Build history of the part. All positions in model axes, mm. A direction names the side the tool comes from. Round coordinates to 2 decimals unless told otherwise and drop trailing zeros. Loops run counter-clockwise (first coordinate to the right, second up) from the corner with the lowest first, then second, coordinate; pieces in that order, holes last. Notation, with made-up numbers: (-19, 67) -> (1, 67) arc R32 cw to (1, 104) -> close; hole circle Ø8 at (75, 46.25). An arc over 180 degrees is marked (long way). Put each result on its own line as item: value. Start each with the question number.
Item 1: Pull direction X, two halves, no side cores. Call faces 1 (the flat face through (-60.136, 53, -48)), 2 (the flat face through (-30.136, 48, -42)), 3 (the cylindrical face through (-15.556, 87.485, -73.11)), 4 (the cylindrical face through (-40, 45.05, -38.12)): +X half, -X half, draft (parallel to the pull), parting line (faces both ways), or undercut.
Item 2: Cut at B-B, the plane y = 87. List the corners of the cut face in (x, z), plus the area to 3 significant figures.
Item 3: Cut at D-D, the plane y = 70. List the corners of the cut face in (x, z), plus the area to 3 significant figures.
Item 4: Drill centre lines: probe 1 along X at (y, z) = (105.5, -31.5); probe 2 along X at (y, z) = (22, -84.5); probe 3 along X at (y, z) = (69, -49). Where is each one in solid material? Low to high. Write a range as [from, to].
Item 5: Tool access for faces 5 (the flat face through (-31.18, 14.42, -89.05)), 6 (the cylindrical face through (-14.926, 82.124, -68.609)), 7 (the cylindrical face through (9.93, 48.87, -41.35)), 8 (the cylindrical face through (-55.066, 61.239, -53.737)), 9 (the cylindrical face through (-15.626, 91.391, -76.232)): list every direction of +Z, -Z, +X, -X, +Y, -Y with a clear straight run to the whole face (end or side of a thin tool).
Item 6: Cut at A-A, the plane x = -40.5. List the corners of the cut face in (y, z), plus the area to 3 significant figures.
Item 7: Flat gauge pins, fed straight in: pin 1 Ø1.5 at (x, z) = (6, -24) entering from -Y; pin 2 Ø4 at (x, z) = (-26.5, -29) entering from +Y; pin 3 Ø10 at (x, z) = (7, -74.5) entering from -Y. Where does each tip first touch, or does it go through?
Item 8: Cut at C-C, the plane z = -96.5. List the corners of the cut face in (x, y), plus the area to 3 significant figures.
```python
from build123d import *

# Parameters (mm, degrees)
REVOLVE1_ANGLE                 = 80
SKETCH3_R                      = 7.5
BOSS_EXTRUDE1_DEPTH            = 10
SHELL3_T                       = -5
CUT_EXTRUDE1_REACH             = 176.812
SKETCH4_R                      = 15
CUT_EXTRUDE1_DIRECTION_2_REACH = 176.812


with BuildPart() as part:
    # Sketch1 → Revolve1 (revolve)
    with BuildSketch(Plane.XY):
        Polygon((-0.136394071, 58.716551136), (19.863605929, 58.716551136), (19.863605929, 118.716551136), (-50.136394071, 118.716551136), (-50.136394071, 58.716551136), (-30.136394071, 58.716551136), (-30.136394071, 106.716551136), (-0.136394071, 106.716551136), align=None)
    revolve(axis=Axis((39.541450035, -1.283448864, 0), (-1, 0, 0)), revolution_arc=REVOLVE1_ANGLE)

    # Sketch3 → Boss-Extrude1 (add)
    with BuildSketch(Plane.ZY.offset(50.136394071)):
        with Locations((-48.209070726, 56.16988437)):
            Circle(SKETCH3_R)
    extrude(amount=BOSS_EXTRUDE1_DEPTH)

    # Shell3
    shell3_openings = [part.faces().sort_by_distance(p)[0] for p in [
        (-60.136394071, 56.16988437, -48.209070726),
    ]]
    offset(amount=SHELL3_T, openings=shell3_openings, kind=Kind.INTERSECTION)

    # Sketch4 → Cut-Extrude1 (cut, up to next)
    with BuildSketch(Plane(origin=(-30.136394071, 0, 0), x_dir=(0, 0, -1), z_dir=(1, 0, 0)), mode=Mode.PRIVATE) as cut_extrude1_sk1:
        with Locations(Location((52.708583994, 61.532195472, 0), (0, 0, 270))):
            Circle(SKETCH4_R)
    cut_extrude1_tool1 = extrude(cut_extrude1_sk1.sketch, amount=-CUT_EXTRUDE1_REACH, mode=Mode.PRIVATE) & part.part
    add(cut_extrude1_tool1.solids().sort_by_distance((-30.136394, 61.532195, -52.708584))[0], mode=Mode.SUBTRACT)

    # Sketch4 → Cut-Extrude1 direction 2 (cut, up to next)
    with BuildSketch(Plane(origin=(-30.136394071, 0, 0), x_dir=(0, 0, -1), z_dir=(1, 0, 0)), mode=Mode.PRIVATE) as cut_extrude1_direction_2_sk1:
        with Locations(Location((52.708583994, 61.532195472, 0), (0, 0, 270))):
            Circle(SKETCH4_R)
    cut_extrude1_direction_2_tool1 = extrude(cut_extrude1_direction_2_sk1.sketch, amount=CUT_EXTRUDE1_DIRECTION_2_REACH, mode=Mode.PRIVATE) & part.part
    add(cut_extrude1_direction_2_tool1.solids().sort_by_distance((-30.136394, 61.532195, -52.708584))[0], mode=Mode.SUBTRACT)


solid = part.part
```
Reply:
1. face 1: -X half
1. face 2: undercut
1. face 3: undercut
1. face 4: draft
2. outline: (-50.14, -81.28) -> (19.86, -81.28) -> (19.86, 0) -> (-0.14, 0) -> (-0.14, -62.21) -> (-30.14, -62.21) -> (-30.14, 0) -> (-50.14, 0) -> close; hole (-45.14, -73.7) -> (14.86, -73.7) -> (14.86, -5) -> (4.86, -5) -> (4.86, -70.53) -> (-35.14, -70.53) -> (-35.14, -5) -> (-45.14, -5) -> close
2. area: 2,320 mm^2
3. outline: (-50.14, -96.53) -> (19.86, -96.53) -> (19.86, 0) -> (-0.14, 0) -> (-0.14, -40.33) -> (4.86, -40.33) -> (4.86, -5) -> (14.86, -5) -> (14.86, -90.24) -> (-45.14, -90.24) -> (-45.14, -5) -> (-35.14, -5) -> (-35.14, -40.33) -> (-30.14, -40.33) -> (-30.14, 0) -> (-50.14, 0) -> close; (-35.14, -87.68) -> (4.86, -87.68) -> (4.86, -65.09) -> (-0.14, -65.09) -> (-0.14, -81.13) -> (-30.14, -81.13) -> (-30.14, -65.09) -> (-35.14, -65.09) -> close
3. area: 2,270 mm^2
4. probe 1: x = [-50.14, -45.14], [-35.14, 4.86], [14.86, 19.86]
4. probe 2: x = [-50.14, -45.14], [-35.14, -30.14], [-0.14, 4.86], [14.86, 19.86]
4. probe 3: x = [-50.14, -45.14], [14.86, 19.86]
5. face 5: -Z, +X, -X, -Y
5. face 6: +Z, -Y
5. face 7: none
5. face 8: -X
5. face 9: -Z, +X, -X, +Y
6. outline: (9.14, -59.09) -> (19.55, -118.18) arc R120 ccw to (118.72, 0) -> (58.72, 0) arc R60 cw to start; hole (14.89, -62.95) -> (23.59, -112.28) arc R115 ccw to (113.61, -5) -> (63.52, -5) arc R65 cw to start
6. area: 1,760 mm^2
7. pin 1: stops at y = 53.37
7. pin 2: stops at y = 115.64
7. pin 3: stops at y = 10.97
8. outline: (-50.14, 15.73) -> (-30.14, 15.73) -> (-30.14, 47.21) -> (-0.14, 47.21) -> (-0.14, 15.73) -> (19.86, 15.73) -> (19.86, 70.05) -> (-50.14, 70.05) -> close; hole (-45.14, 20.81) -> (-35.14, 20.81) -> (-35.14, 57.51) -> (4.86, 57.51) -> (4.86, 20.81) -> (14.86, 20.81) -> (14.86, 61.27) -> (-45.14, 61.27) -> close
8. area: 1,900 mm^2
